from build123d import *

# Parameters (mm, degrees)
SKETCH_1_R             = 10
EXTRUDE_1_DEPTH        = 113.5
SKETCH_2_W             = 0.5
SKETCH_2_H             = 1.1
CHAMFER_1_SIZE         = 1
HOLE_WIZARD_M6_1_D     = 5
HOLE_WIZARD_M6_1_DEPTH = 21


with BuildPart() as part:
    # 草图1 → 凸台-拉伸1 (new body)
    with BuildSketch(Plane.XY):
        with Locations(Location((0, 0, 0), (0, 0, 180))):
            Circle(SKETCH_1_R)
    extrude(amount=EXTRUDE_1_DEPTH)

    # 草图2 → 切除-旋转1 (revolve, cut)
    with BuildSketch(Plane(origin=(0, 0, 0), x_dir=(1, 0, 0), z_dir=(0, 1, 0)), mode=Mode.PRIVATE) as cut_revolve_1_sk:
        with Locations((9.75, -108.95)):
            Rectangle(SKETCH_2_W, SKETCH_2_H)
    revolve(cut_revolve_1_sk.sketch.rotate(Axis((0, 0, 113.5), (0, 0, -1)), 180), axis=Axis((0, 0, 113.5), (0, 0, -1)), mode=Mode.SUBTRACT)

    # 倒角1
    chamfer_1_edges = [part.edges().sort_by_distance(p)[0] for p in [
        (10, 0, 0),
        (10, 0, 113.5),
    ]]
    chamfer(chamfer_1_edges, length=CHAMFER_1_SIZE)

    # M6 螺纹孔1
    with Locations(Plane(origin=(0, 0, 0), x_dir=(-1, 0, 0), z_dir=(0, 0, -1))):
        with Locations((0, 0)):
            Hole(HOLE_WIZARD_M6_1_D / 2, depth=HOLE_WIZARD_M6_1_DEPTH)


solid = part.part
Geometry: final body of the model. Coordinates: model frame, mm. A direction names the side the tool comes from. Round coordinates to 2 decimals unless told otherwise and drop trailing zeros. Loops run counter-clockwise (first coordinate to the right, second up) from the corner with the lowest first, then second, coordinate; pieces in that order, holes last. Notation, with made-up numbers: M -20.75,-36 L -7.75,-36 A27 ccw -7.75,-9 Z; hole C 75,39 d7. An arc over 180 degrees is marked long. One line per question, with ' | ' between items.
(1) Pull-direction query (Z, two-part tool) for faces 4 (the cylindrical face through (10, 0, 54)), 5 (the flat face through (-2, 2, 0)), 6 (the cylindrical face through (2.059, -9.274, 108.942)); classes: +Z half, -Z half, draft (parallel to the pull), parting line (faces both ways), or undercut.
Check result:
face 4: draft | face 5: -Z half | face 6: undercut
(2) Cut plane B-B on z = 8.5. Return the cut outline in (x, y), plus the area to 3 significant figures.
Check result:
outline: C 0,0 d20; hole C 0,0 d5 | area: 295 mm2
(3) Access query for faces 1 (the cylindrical face through (-0.54, -2.44, 10.65)), 2 (the cylindrical face through (10, 0, 111)), 3 (the flat face through (9, -4, 108.4)). Directions: +Z, -Z, +X, -X, +Y, -Y. A direction counts if a zero-diameter tool reaches every point of the face in a straight line with its end or side. Return the directions, or none.
Check result:
face 1: -Z | face 2: +Z, -Z | face 3: none
(4) Cut plane D-D on z = 39.5. Return the cut outline in (x, y).
Check result:
outline: C 0,0 d20
(5) Contact query for flat-ended pins moving along their axis: P1, Ø3, axis at y = 6.5, z = 78, coming from the +X side; P2, Ø1.5, axis at x = -7, z = 71.5, coming from the +Y side; P3, Ø1.5, axis at x = -0.5, y = 0, coming from the -Z side. Output: stop coordinate, or through.
Check result:
P1: stops at x = 8.66 | P2: stops at y = 7.81 | P3: stops at z = 21
(6) Cut plane A-A on x = 0. Return the cut outline in (y, z).
Check result:
outline: M -10,1 L -9,0 L -2.5,0 L -2.5,21 L 2.5,21 L 2.5,0 L 9,0 L 10,1 L 10,108.4 L 9.5,108.4 L 9.5,109.5 L 10,109.5 L 10,112.5 L 9,113.5 L -9,113.5 L -10,112.5 L -10,109.5 L -9.5,109.5 L -9.5,108.4 L -10,108.4 Z
(7) Material intervals for line 1 along Y through (x, z) = (0, 14); line 2 along Y through (x, z) = (-0.25, 50); line 3 along X through (y, z) = (2.25, 90), sorted ascending. Write a range as from..to.
Check result:
line 1: y = -10..-2.5, 2.5..10 | line 2: y = -10..10 | line 3: x = -9.74..9.74
